Read the model definition and answer for the solid it produces. Units are mm, in the model's axes. A direction names the side the tool comes from. Coordinates: 2 decimals unless noted, no trailing zeros. Order: outer loops, then holes, each group sorted by start corner. A loop starts at its lowest first (then second) coordinate and runs counter-clockwise, first axis right, second up. Notation, with made-up numbers: (2, 83.25) -> (8, 83.25) arc R28 ccw to (8, 104.25) -> close; hole circle Ø4 at (86, -36). An arc over 180 degrees is marked (long way). Answer in a Markdown table with one row per item.
from build123d import *

# Parameters (mm, degrees)
PIN_BORE_SKETCH_R         = 10
GUDGEON_PIN_BORE_20_DEPTH = 66
EDGE_CHAMFER_2X45_SIZE    = 2
INNER_CAVITY_SKETCH_W     = 20
INNER_CAVITY_SKETCH_H     = 29
INNER_CAVITY_CUT_DEPTH    = 48


with BuildPart() as part:
    # Piston Profile Sketch → Piston Body Revolve (revolve)
    with BuildSketch(Plane.XY, mode=Mode.PRIVATE) as piston_body_revolve_sk:
        Polygon((-24, 0), (-30, 0), (-30, 48), (-27, 48), (-27, 51), (-30, 51), (-30, 54), (-27, 54), (-27, 57), (-30, 57), (-30, 60), (-27, 60), (-27, 63), (-30, 63), (-30, 66), (-27, 66), (-27, 69), (-30, 69), (-30, 72), (0, 72), (0, 60), (-24, 60), (-24, 48), (-10, 48), (-10, 22), (-24, 22), align=None)
    revolve(piston_body_revolve_sk.sketch.rotate(Axis((0, 60, 0), (0, 1, 0)), 180), axis=Axis((0, 60, 0), (0, 1, 0)))

    # Pin Bore Sketch → Gudgeon Pin Bore Ø20 (cut, symmetric)
    with BuildSketch(Plane(origin=(0, 0, 0), x_dir=(0, 0, -1), z_dir=(1, 0, 0))):
        with Locations(Location((0, 35, 0), (0, 0, 270))):
            Circle(PIN_BORE_SKETCH_R)
    extrude(amount=GUDGEON_PIN_BORE_20_DEPTH, both=True, mode=Mode.SUBTRACT)

    # Edge Chamfer 2x45°
    edge_chamfer_2x45_edges = [part.edges().sort_by_distance(p)[0] for p in [
        (-24, 0, 0),
    ]]
    chamfer(edge_chamfer_2x45_edges, length=EDGE_CHAMFER_2X45_SIZE)

    # Inner Cavity Sketch → Inner Cavity Cut (cut)
    with BuildSketch(Plane.XZ):
        Rectangle(INNER_CAVITY_SKETCH_W, INNER_CAVITY_SKETCH_H)
    extrude(amount=-INNER_CAVITY_CUT_DEPTH, mode=Mode.SUBTRACT)


solid = part.part
Q1. The part is cut by section A-A (y = 31.5). Write down the section's boundary in (x, z).
Outcome:
| item | result |
|---|---|
| outline | (-28.5, -9.37) arc R30 ccw to (28.5, -9.37) -> (10, -9.37) -> (10, -14.5) -> (-10, -14.5) -> (-10, -9.37) -> close; (-28.5, 9.37) -> (-10, 9.37) -> (-10, 14.5) -> (10, 14.5) -> (10, 9.37) -> (28.5, 9.37) arc R30 ccw to start |
Q2. For a pull along Z with two mould halves and no side action, classify faces 1 (the face through (0, 60, 0)), 2 (the face through (25, 69, -11)), 3 (the face through (-5.85, 49.52, 26.36)) as pulls with the +Z half, pulls with the -Z half, needs draft (parallel to the pull), parting line crosses it, or undercut.
Outcome:
| item | result |
|---|---|
| face 1 | undercut |
| face 2 | needs draft |
| face 3 | parting line crosses it |
Q3. For faces 4 (the face through (-5.85, 67.52, 26.36)), 5 (the face through (16.128, 52.521, -25.296)), 6 (the face through (0, 35, 14.5)), determine the directions among +Z, -Z, +X, -X, +Y, -Y from which every point of the face is accessible in a straight line to the end or side of a thin tool.
Outcome:
| item | result |
|---|---|
| face 4 | none |
| face 5 | +Y, -Y |
| face 6 | -Y |
Q4. Given pin 1 (16 mm diameter, centred on x = -4, y = 39, fed in from -Z); pin 2 (2 mm diameter, centred on x = 10.5, y = 40, fed in from -Z); pin 3 (8 mm diameter, centred on y = 41, z = 1, fed in from -X); pin 4 (8 mm diameter, centred on y = 38, z = -3, fed in from +X), each flat-ended and moving along its own axis, determine where each tip first touches the part or whether it passes through.
Outcome:
| item | result |
|---|---|
| pin 1 | z = -30 |
| pin 2 | z = -28.46 |
| pin 3 | x = -29.99 |
| pin 4 | through |
Q5. Consider line 1 (Z direction, x = 0, y = 57.5); line 2 (Y direction, x = -0.5, z = -15); line 3 (Y direction, x = 14, z = -4). Determine where each line is inside the solid, lowest interval first.
Outcome:
| item | result |
|---|---|
| line 1 | -30 to -24, 24 to 30 |
| line 2 | 22 to 48, 60 to 72 |
| line 3 | 22 to 25.83, 44.17 to 48, 60 to 72 |
Q6. The part is cut by section C-C (z = 0). Give the number of separate pieces and of enclosed holes in the cut face, then the cut area to 3 significant figures.
Outcome:
| item | result |
|---|---|
| separate pieces | 3 |
| enclosed holes | 0 |
| area | 1,290 mm² |
Q7. The part is cut by section B-B (y = 9.5). Write down the section's boundary in (x, z).
Outcome:
| item | result |
|---|---|
| outline | circle Ø60 at (0, 0); hole circle Ø48 at (0, 0) |
Q8. The part is cut by section D-D (y = 43). Write down the section's boundary in (x, z), then the cut area to 3 significant figures.
Outcome:
| item | result |
|---|---|
| outline | (-29.39, -6) arc R30 ccw to (29.39, -6) -> (10, -6) -> (10, -14.5) -> (-10, -14.5) -> (-10, -6) -> close; (-29.39, 6) -> (-10, 6) -> (-10, 14.5) -> (10, 14.5) -> (10, 6) -> (29.39, 6) arc R30 ccw to start |
| area | 1,770 mm² |
